Part model, mm, in its own coordinate system. Coordinates: 2 decimals unless noted, no trailing zeros. Loops run counter-clockwise (first coordinate to the right, second up) from the corner with the lowest first, then second, coordinate; pieces in that order, holes last. Notation, with made-up numbers: (-26, 47) - (9, 47) arc R18 ccw to (9, 81) - close; hole circle Ø2 at (-22, 62). An arc over 180 degrees is marked (long way). Answer as CSV lines item,"result".
from build123d import *

# Parameters (mm, degrees)
LINK_BAR_PROFILE_R  = 25
LINK_BAR_20MM_DEPTH = 20


with BuildPart() as part:
    # Link Bar Profile → Link Bar 20mm (new body)
    with BuildSketch(Plane.XY):
        with BuildLine():
            Line((-50, 0), (-50, 255))
            ThreePointArc((-50, 255), (0, 305), (50, 255))
            Line((50, 255), (50, 0))
            ThreePointArc((50, 0), (0, -50), (-50, 0))
        make_face()
        with Locations((0, 255)):
            Circle(LINK_BAR_PROFILE_R, mode=Mode.SUBTRACT)
        Circle(LINK_BAR_PROFILE_R, mode=Mode.SUBTRACT)
    extrude(amount=LINK_BAR_20MM_DEPTH)


solid = part.part
Q1. Saw through at B-B (y = 8). Give the cut face in (x, z), then the cut area to 3 significant figures.
Results:
outline,"(-50, 0) - (-23.69, 0) - (-23.69, 20) - (-50, 20) - close; (23.69, 0) - (50, 0) - (50, 20) - (23.69, 20) - close"
area,"1,050 mm^2"
Q2. Saw through at C-C (z = 15.5). Give the cut face in (x, y).
Results:
outline,"(-50, 0) arc R50 ccw to (50, 0) - (50, 255) arc R50 ccw to (-50, 255) - close; hole circle Ø50 at (0, 0); hole circle Ø50 at (0, 255)"
Q3. Two-plate mould, pull along X, no slides. Class faces 1 (the face through (-3.255, 279.787, 9.86)), 2 (the face through (-1.099, 304.988, 9.86)), 3 (the face through (1, 130, 0)), 4 (the face through (-50, 126, 10)): released by +X, released by -X, zero draft, split by the parting line, or undercut.
Results:
face 1,"undercut"
face 2,"split by the parting line"
face 3,"zero draft"
face 4,"released by -X"
Q4. Saw through at A-A (x = 0). Give the cut face in (y, z), then the cut area to 3 significant figures.
Results:
outline,"(-50, 0) - (-25, 0) - (-25, 20) - (-50, 20) - close; (25, 0) - (230, 0) - (230, 20) - (25, 20) - close; (280, 0) - (305, 0) - (305, 20) - (280, 20) - close"
area,"5,100 mm^2"
Q5. Wall check: L1, parallel to Y at x = 0, z = 10; L2, parallel to Y at x = -9, z = 2.5; L3, parallel to X at y = 8.5, z = 3. Give the ranges that are in metal, low to high.
Results:
L1,"y = -50 to -25, 25 to 230, 280 to 305"
L2,"y = -49.18 to -23.32, 23.32 to 231.68, 278.32 to 304.18"
L3,"x = -50 to -23.51, 23.51 to 50"
Q6. Flat gauge pins, fed straight in: pin 1 (4 mm diameter, centred on x = 32, z = 3, fed in from +Y); pin 2 (5 mm diameter, centred on x = -16.5, z = 9.5, fed in from -Y); pin 3 (3 mm diameter, centred on x = -11, z = 14.5, fed in from -Y). Where does each tip first touch, or does it go through?
Results:
pin 1,"stops at y = 295"
pin 2,"stops at y = -48"
pin 3,"stops at y = -49.09"
